Drawing for the job (mm, zero at the part's lowest x, y, z). A direction names the side the tool comes from. Round coordinates to 2 decimals unless told otherwise and drop trailing zeros. Order: outer loops, then holes, each group sorted by start corner. A loop starts at its lowest first (then second) coordinate and runs counter-clockwise, first axis right, second up. Notation, with made-up numbers: (45, 47) - (55, 47) arc R36 ccw to (55, 85) - close; hole circle Ø10 at (-19, -21). An arc over 180 degrees is marked (long way). Put each result on its own line as item: value. Start each with the question number.
Item 1: Saw through at B-B on y = 6. List the corners of the cut face in (x, z).
Item 2: Saw through at D-D on x = 16.75. List the corners of the cut face in (y, z).
Item 3: Which spindle directions (+Z, -Z, +X, -X, +Y, -Y) get a long thin tool onto all of the face, cutting with end or side? Do the marked faces 1 and 2. Say none if no direction does.
Item 4: Saw through at A-A on x = 9.55. List the corners of the cut face in (y, z).
Item 5: Probe probe 1 along Z at (x, y) = (7.75, 6.5); probe 2 along Y at (x, z) = (11.25, 5.25); probe 3 along X at (y, z) = (6.5, 2). List the from-to ranges inside material, lowest first.
Item 6: Mould opens along Z. For the marked faces 3, 4 and 5 say: pulls with the +Z half, pulls with the -Z half, needs draft (parallel to the pull), parting line crosses it, or undercut.
Item 7: Pin check, flat tips, straight feed: pin 1 Ø2 at (x, y) = (14.47, 6) entering from -Z; pin 2 Ø4 at (x, y) = (3, 8) entering from +Z; pin 3 Ø5.5 at (x, z) = (8, 6) entering from +Y. Stop position of each tip, or through.
Item 8: Saw through at C-C on z = 7.5. List the corners of the cut face in (x, y) (1 decimal).
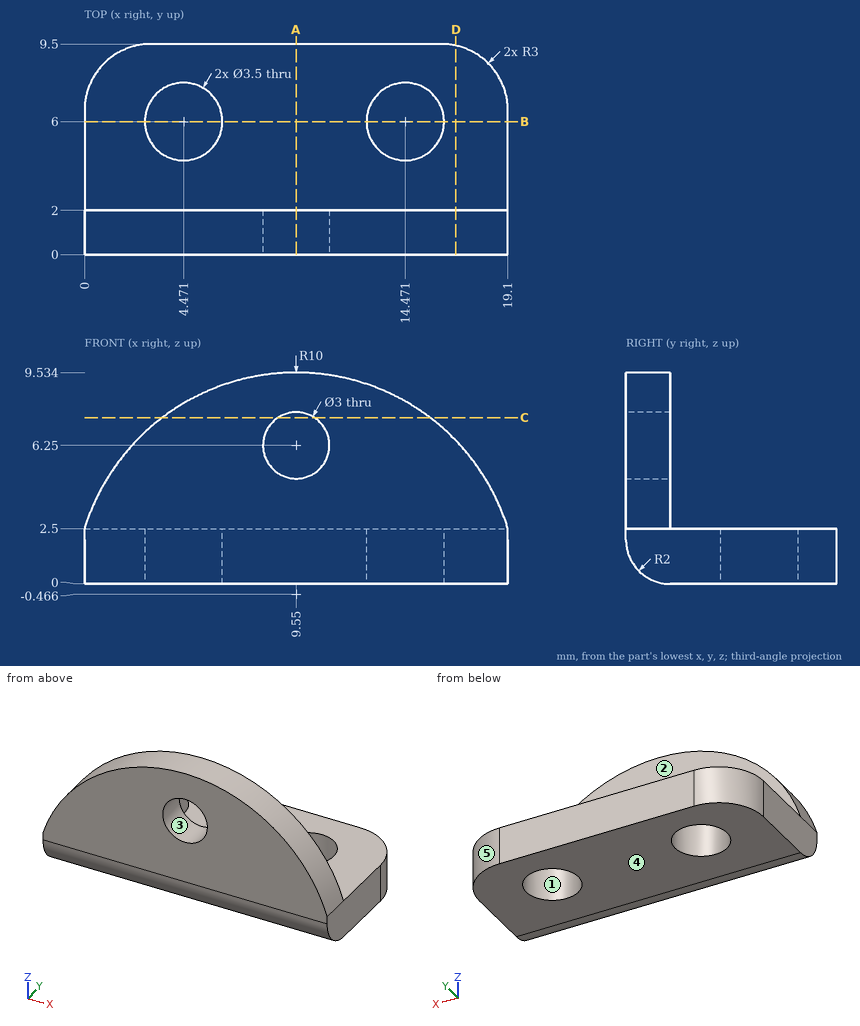
Results found:
1. outline: (0, 0) - (2.72, 0) - (2.72, 2.5) - (0, 2.5) - close; (6.22, 0) - (12.72, 0) - (12.72, 2.5) - (6.22, 2.5) - close; (16.22, 0) - (19.1, 0) - (19.1, 2.5) - (16.22, 2.5) - close
2. outline: (0, 2) arc R2 ccw to (2, 0) - (9.43, 0) - (9.43, 2.5) - (2, 2.5) - (2, 6.47) - (0, 6.47) - close
3. face 1: +Z, -Z
3. face 2: +Z, +X, -X, +Y
4. outline: (0, 2) arc R2 ccw to (2, 0) - (9.5, 0) - (9.5, 2.5) - (2, 2.5) - (2, 4.75) - (0, 4.75) - close; (0, 7.75) - (2, 7.75) - (2, 9.53) - (0, 9.53) - close
5. probe 1: z = 0 to 2.5
5. probe 2: y = 0 to 2
5. probe 3: x = 0 to 2.79, 6.15 to 12.79, 16.15 to 19.1
6. face 3: undercut
6. face 4: pulls with the -Z half
6. face 5: needs draft
7. pin 1: passes through
7. pin 2: stops at z = 2.5
7. pin 3: stops at y = 2
8. outline: (3.5, 0) - (8.7, 0) - (8.7, 2) - (3.5, 2) - close; (10.4, 0) - (15.6, 0) - (15.6, 2) - (10.4, 2) - close
